Source: CAD feature listing. Evaluate the final solid. Frame: model axes, mm. A direction names the side the tool comes from. Round coordinates to 2 decimals unless told otherwise and drop trailing zeros. Order: outer loops, then holes, each group sorted by start corner. A loop starts at its lowest first (then second) coordinate and runs counter-clockwise, first axis right, second up. Notation, with made-up numbers: (-15, 71) - (18, 71) arc R27 ccw to (18, 87) - close; hole circle Ø8 at (-8.75, -28.75). An arc over 180 degrees is marked (long way). Use one line per item in the form item = value. Start each with the question number.
Q1. Set-up query: faces 4 (the flat face through (-83, -60, 6)), 5 (the cylindrical face through (-93.41, -50.44, 6.54)), 6 (the cylindrical face through (-46.59, 4.751, 8.385)). Return all of +Z, -Z, +X, -X, +Y, -Y with unobstructed straight access to the full face (end or side cutting, diameter ignored); none if empty.
Q2. Cut plane D-D, the plane x = -59.5. Return the cut outline in (y, z).
Q3. Cut plane B-B, the plane x = -92. Return the cut outline in (y, z).
Q4. Draft query along Y for faces 1 (the flat face through (-53, -44, 6)), 2 (the cylindrical face through (-46.59, -18.22, 7.15)), 3 (the flat face through (-70, -23, 0)). Return one class per face: released by +Y, released by -Y, zero draft, split by the parting line, or undercut.
Q5. Cut plane A-A, the plane z = 9.5. Return the cut outline in (x, y).
Q6. Cut plane C-C, the plane y = -52.5. Return the cut outline in (x, z).
Q7. Ray query, line 1 (Z direction, x = -93, y = -48); line 2 (Y direction, x = -43.5, z = 7.5); line 3 (Y direction, x = -90.25, z = 6). Return the intervals inside material, ascending. Write a range as [from, to].
from build123d import *

# Parameters (mm, degrees)
EXTRUDE_1_DEPTH        = 12
CHAMFER_1_SIZE         = 10
HOLE_WIZARD_M6_1_D     = 5
HOLE_WIZARD_M6_1_DEPTH = 13
HOLE_WIZARD_M6_1_TIP   = 1.502151548
HOLE_WIZARD_M6_2_D     = 5
HOLE_WIZARD_M6_2_DEPTH = 13
HOLE_WIZARD_M6_2_TIP   = 1.502151548


with BuildPart() as part:
    # 草图1 → 凸台-拉伸1 (new body)
    with BuildSketch(Plane.XY):
        Polygon((-39.998611317, 12), (-39.998611317, -28), (-65.998611317, -60), (-99.998611317, -60), (-99.998611317, 12), align=None)
    extrude(amount=EXTRUDE_1_DEPTH)

    # 倒角1
    chamfer_1_edges = [part.edges().sort_by_distance(p)[0] for p in [
        (-99.998611317, 12, 6),
    ]]
    chamfer(chamfer_1_edges, length=CHAMFER_1_SIZE)

    # M6 螺纹孔1
    with Locations(Plane(origin=(-39.998611317, 0, 0), x_dir=(0, 0, -1), z_dir=(1, 0, 0))):
        with Locations((-6, 4), (-6, -16)):
            Hole(HOLE_WIZARD_M6_1_D / 2, depth=HOLE_WIZARD_M6_1_DEPTH)
            with Locations((0, 0, -(HOLE_WIZARD_M6_1_DEPTH + HOLE_WIZARD_M6_1_TIP / 2))):  # 118° drill point
                Cone(0, HOLE_WIZARD_M6_1_D / 2, HOLE_WIZARD_M6_1_TIP, mode=Mode.SUBTRACT)

    # M6 螺纹孔2
    with Locations(Plane.ZY.offset(99.998611317)):
        with Locations((6, -8), (6, -48)):
            Hole(HOLE_WIZARD_M6_2_D / 2, depth=HOLE_WIZARD_M6_2_DEPTH)
            with Locations((0, 0, -(HOLE_WIZARD_M6_2_DEPTH + HOLE_WIZARD_M6_2_TIP / 2))):  # 118° drill point
                Cone(0, HOLE_WIZARD_M6_2_D / 2, HOLE_WIZARD_M6_2_TIP, mode=Mode.SUBTRACT)


solid = part.part
Completed:
q1.face_4 = +Z, -Z, +X, -X, -Y
q1.face_5 = -X
q1.face_6 = +X
q2.outline = (-52, 0) - (12, 0) - (12, 12) - (-52, 12) - close
q3.outline = (-60, 0) - (10, 0) - (10, 12) - (-60, 12) - close; hole circle Ø5 at (-48, 6); hole circle Ø5 at (-8, 6)
q4.face_1 = released by -Y
q4.face_2 = undercut
q4.face_3 = zero draft
q5.outline = (-100, -60) - (-66, -60) - (-40, -28) - (-40, 12) - (-90, 12) - (-100, 2) - close
q6.outline = (-100, 0) - (-59.9, 0) - (-59.9, 12) - (-100, 12) - close
q7.line_1 = [0, 3.5], [8.5, 12]
q7.line_2 = [-32.31, -18], [-14, 2], [6, 12]
q7.line_3 = [-60, -50.5], [-45.5, -10.5], [-5.5, 11.75]
